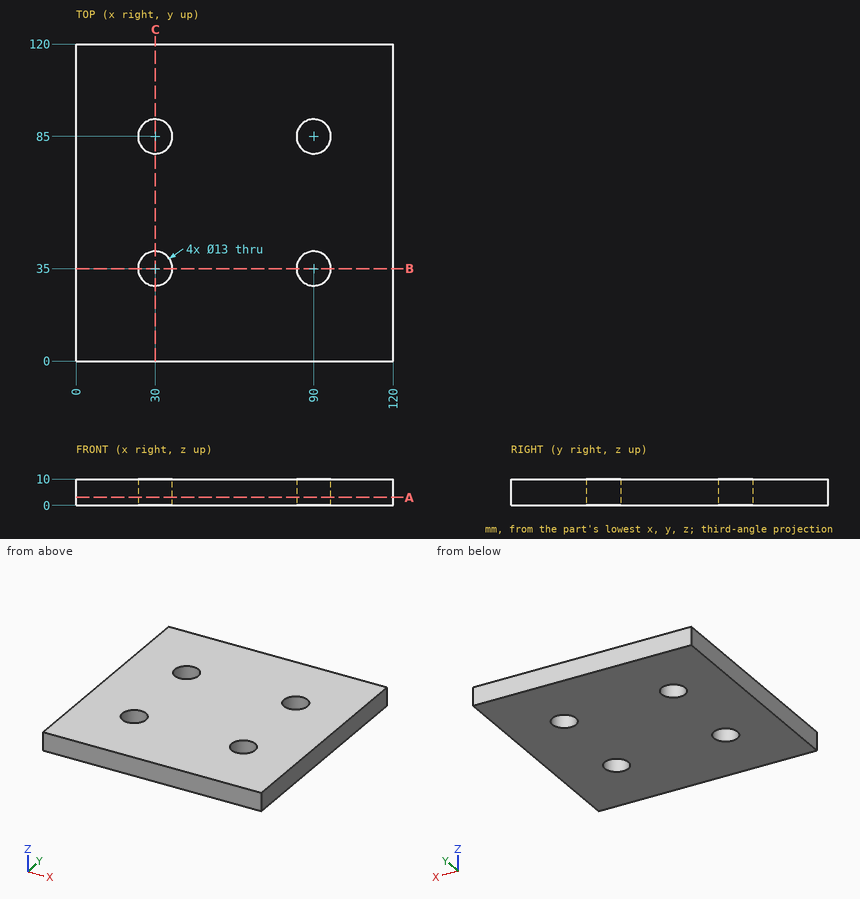
For this review, use the dimensioned drawing (mm, ordinates from the lowest corner) and the shaded views. Give positions to 0.01 mm unless a question says otherwise; leave off trailing zeros. Loops run counter-clockwise (first coordinate to the right, second up) from the corner with the lowest first, then second, coordinate; pieces in that order, holes last.
Item 1: Take a section at B-B, the plane y = 35. State the section outline as (x, z) points, and give its area (3 significant figures).
Item 2: Insertion check: pin 1 (11.5 mm diameter, centred on x = 90, y = 35, fed in from +Z). The pin has a flat end and moves straight along its axis. Give the tip position at first contact, or say it passes through.
Item 3: For line 1 along Y through (x, z) = (90, 7.75); line 2 along Y through (x, z) = (87, 1.25); line 3 along X through (y, z) = (34, 7), list the stretches that pass through material, from the lowest coordinate up.
Item 4: Take a section at A-A, the plane z = 3. State the section outline as (x, y) points.
Item 5: Take a section at C-C, the plane x = 30. State the section outline as (y, z) points.
Calculated:
1. outline: (0, 0) - (23.5, 0) - (23.5, 10) - (0, 10) - close; (36.5, 0) - (83.5, 0) - (83.5, 10) - (36.5, 10) - close; (96.5, 0) - (120, 0) - (120, 10) - (96.5, 10) - close
1. area: 940 mm2
2. pin 1: passes through
3. line 1: y = 0 to 28.5, 41.5 to 78.5, 91.5 to 120
3. line 2: y = 0 to 29.23, 40.77 to 79.23, 90.77 to 120
3. line 3: x = 0 to 23.58, 36.42 to 83.58, 96.42 to 120
4. outline: (0, 0) - (120, 0) - (120, 120) - (0, 120) - close; hole circle Ø13 at (30, 35); hole circle Ø13 at (30, 85); hole circle Ø13 at (90, 35); hole circle Ø13 at (90, 85)
5. outline: (0, 0) - (28.5, 0) - (28.5, 10) - (0, 10) - close; (41.5, 0) - (78.5, 0) - (78.5, 10) - (41.5, 10) - close; (91.5, 0) - (120, 0) - (120, 10) - (91.5, 10) - close
